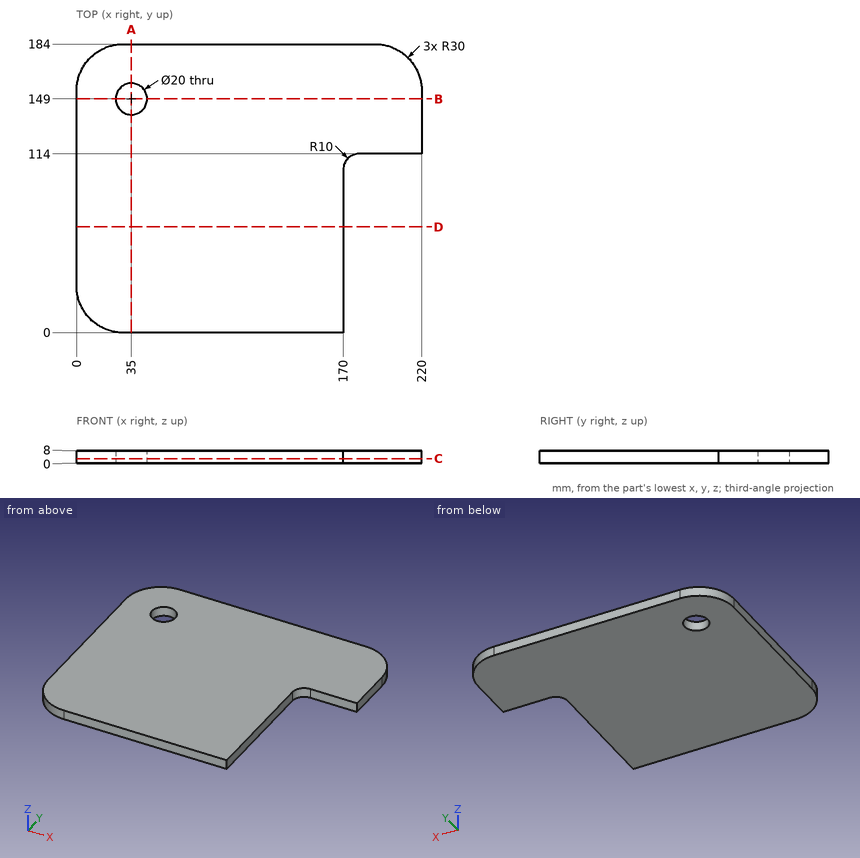
Verification items for this drawing (mm, ordinates from the low corner). Round coordinates to 2 decimals unless told otherwise and drop trailing zeros. Loops run counter-clockwise (first coordinate to the right, second up) from the corner with the lowest first, then second, coordinate; pieces in that order, holes last. Notation, with made-up numbers: (48.5, 43.5) - (77.5, 43.5) arc R20 cw to (77.5, 56.5) - close; hole circle Ø5 at (8, 27). An arc over 180 degrees is marked (long way). Answer as CSV lines item,"result". Start each with the question number.
Item 1: Scan lines: line 1 (Y direction, x = 35, z = 5.75); line 2 (X direction, y = 142.5, z = 5.5); line 3 (X direction, y = 156.5, z = 6.25). Record each from-to range of solid material in increasing order. Write a range as [from, to].
Item 2: Section check B-B (y = 149). Record the boundary of the cut face in (x, z), and give its area (3 significant figures).
Item 3: Section check C-C (z = 3). Record the boundary of the cut face in (x, y), and give its area (3 significant figures).
Item 4: Section check D-D (y = 67.5). Record the boundary of the cut face in (x, z).
Item 5: Depth check by flat-ended pin: P1, Ø4, axis at y = 65.5, z = 4, coming from the +X side; P2, Ø2.5, axis at x = 208, z = 4, coming from the -Y side; P3, Ø4, axis at x = 197.5, z = 3, coming from the +Y side. Enter the tip coordinate at first touch or a pass-through.
Item 6: Section check A-A (x = 35). Record the boundary of the cut face in (y, z).
Report:
1,line 1,"y = [0, 139], [159, 184]"
1,line 2,"x = [0, 27.4], [42.6, 220]"
1,line 3,"x = [0.1, 28.39], [41.61, 219.9]"
2,outline,"(0, 0) - (25, 0) - (25, 8) - (0, 8) - close; (45, 0) - (220, 0) - (220, 8) - (45, 8) - close"
2,area,"1,600 mm2"
3,outline,"(0, 30) arc R30 ccw to (30, 0) - (170, 0) - (170, 104) arc R10 cw to (180, 114) - (220, 114) - (220, 154) arc R30 ccw to (190, 184) - (30, 184) arc R30 ccw to (0, 154) - close; hole circle Ø20 at (35, 149)"
3,area,"33,900 mm2"
4,outline,"(0, 0) - (170, 0) - (170, 8) - (0, 8) - close"
5,P1,"stops at x = 170"
5,P2,"stops at y = 114"
5,P3,"stops at y = 183.49"
6,outline,"(0, 0) - (139, 0) - (139, 8) - (0, 8) - close; (159, 0) - (184, 0) - (184, 8) - (159, 8) - close"
